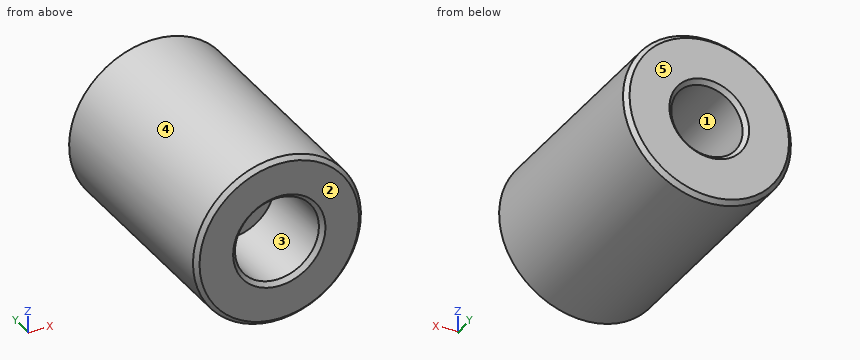
```python
from build123d import *

# Parameters (mm, degrees)
SKETCH_1_R          = 20
EXTRUDE_1_DEPTH     = 55
SKETCH_2_R          = 8.5
CUT_EXTRUDE_1_DEPTH = 20
SKETCH_3_R          = 10
CUT_EXTRUDE_2_DEPTH = 20
CHAMFER_1_SIZE      = 1


with BuildPart() as part:
    # 草图1 → 凸台-拉伸1 (new body)
    with BuildSketch(Plane(origin=(0, 0, 0), x_dir=(1, 0, 0), z_dir=(0, 1, 0))):
        with Locations(Location((0, 0, 0), (0, 0, 270))):
            Circle(SKETCH_1_R)
    extrude(amount=EXTRUDE_1_DEPTH)

    # 草图2 → 切除-拉伸1 (cut)
    with BuildSketch(Plane(origin=(0, 55, 0), x_dir=(1, 0, 0), z_dir=(0, 1, 0))):
        with Locations(Location((0, 0, 0), (0, 0, 270))):
            Circle(SKETCH_2_R)
    extrude(amount=-CUT_EXTRUDE_1_DEPTH, mode=Mode.SUBTRACT)

    # 草图3 → 切除-拉伸2 (cut)
    with BuildSketch(Plane.XZ):
        with Locations(Location((0, 0, 0), (0, 0, 270))):
            Circle(SKETCH_3_R)
    extrude(amount=-CUT_EXTRUDE_2_DEPTH, mode=Mode.SUBTRACT)

    # 倒角1
    chamfer_1_edges = [part.edges().sort_by_distance(p)[0] for p in [
        (0, 0, 10),
        (0, 0, -20),
        (0, 55, -20),
        (0, 55, -8.5),
    ]]
    chamfer(chamfer_1_edges, length=CHAMFER_1_SIZE)


solid = part.part
```
Geometry: final body of the model. Coordinates: model frame, mm. Face numbers are marked on the shaded views. A direction names the side the tool comes from. Round coordinates to 2 decimals unless told otherwise and drop trailing zeros. Order: outer loops, then holes, each group sorted by start corner. A loop starts at its lowest first (then second) coordinate and runs counter-clockwise, first axis right, second up. Notation, with made-up numbers: (-12, 12.5) - (3, 12.5) arc R20 cw to (3, 39.5) - close; hole circle Ø9 at (72, -19.75). An arc over 180 degrees is marked (long way). Use CSV: the item, a comma, the result in double quotes. Start each with the question number.
Q1. Material intervals for line 1 along X through (y, z) = (48.75, 0); line 2 along X through (y, z) = (42, -2); line 3 along Z through (x, y) = (8, 17), sorted ascending. Write a range as from..to.
Q2. Section query D-D (y = 32.5). Return loops of the section in (x, z), and give its area (3 significant figures).
Q3. Section query C-C (y = 43). Return loops of the section in (x, z), and give its area (3 significant figures).
Q4. Access query for the marked faces 1 and 2. Directions: +Z, -Z, +X, -X, +Y, -Y. A direction counts if a zero-diameter tool reaches every point of the face in a straight line with its end or side. Return the directions, or none.
Q5. Mould query, pull axis Z, two halves, no side actions, for the marked faces 3, 4 and 5. Classes: +Z half, -Z half, draft (parallel to the pull), parting line (faces both ways), or undercut.
Q6. Section query B-B (x = 0). Return loops of the section in (y, z), and give its area (3 significant figures).
Q7. First-contact query: pin 1 (10 mm diameter, centred on x = -6.5, y = 11, fed in from +Z); pin 2 (3 mm diameter, centred on y = 45, z = -7.5, fed in from -X); pin 3 (3 mm diameter, centred on y = 41.5, z = -6.5, fed in from +X). Flat tips, straight axial feed; report the tip coordinate or a pass-through.
Q8. Section query A-A (z = 0). Return loops of the section in (x, y), and give its area (3 significant figures).
Result set:
1,line 1,"x = -20..-8.5, 8.5..20"
1,line 2,"x = -19.9..-8.26, 8.26..19.9"
1,line 3,"z = -18.33..-6, 6..18.33"
2,outline,"circle Ø40 at (0, 0)"
2,area,"1,260 mm2"
3,outline,"circle Ø40 at (0, 0); hole circle Ø17 at (0, 0)"
3,area,"1,030 mm2"
4,face 1,"+Y"
4,face 2,"+Z, -Z, +X, -X, -Y"
5,face 3,"undercut"
5,face 4,"parting line"
5,face 5,"draft"
6,outline,"(0, -19) - (1, -20) - (54, -20) - (55, -19) - (55, -9.5) - (54, -8.5) - (35, -8.5) - (35, 8.5) - (54, 8.5) - (55, 9.5) - (55, 19) - (54, 20) - (1, 20) - (0, 19) - (0, 11) - (1, 10) - (20, 10) - (20, -10) - (1, -10) - (0, -11) - close"
6,area,"1,460 mm2"
7,pin 1,"stops at z = 19.94"
7,pin 2,"stops at x = -19.08"
7,pin 3,"stops at x = 19.36"
8,outline,"(-20, 1) - (-19, 0) - (-11, 0) - (-10, 1) - (-10, 20) - (10, 20) - (10, 1) - (11, 0) - (19, 0) - (20, 1) - (20, 54) - (19, 55) - (9.5, 55) - (8.5, 54) - (8.5, 35) - (-8.5, 35) - (-8.5, 54) - (-9.5, 55) - (-19, 55) - (-20, 54) - close"
8,area,"1,460 mm2"
